The listing builds one solid part. Answer for the finished solid, in the listing's coordinates (mm). Give positions to 0.01 mm unless a question says otherwise; leave off trailing zeros. Write each loop counter-clockwise with the first axis right and the second up, starting at its lowest first coordinate (ties: lowest second). Pieces come first, ordered by that corner, then holes. Notation, with made-up numbers: (-19, -37.75) - (27, -37.75) arc R10 cw to (27, -23.75) - close; hole circle Ø7 at (-1, 52.25). An arc over 180 degrees is marked (long way). Return JSON: item names as keys, results as strings.
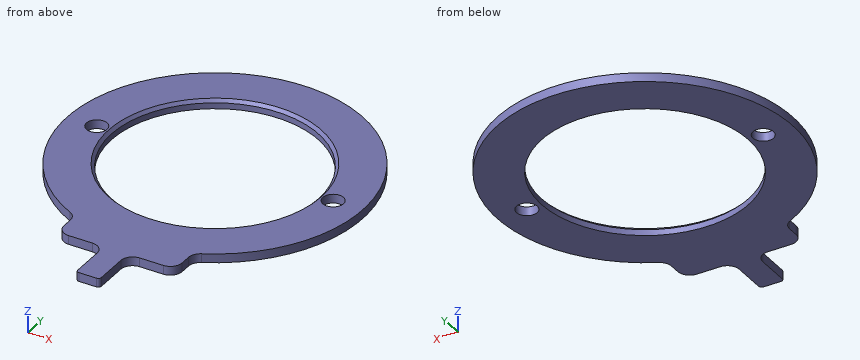
from build123d import *

# Parameters (mm, degrees)
SKETCH_1_R          = 25
SKETCH_1_R_2        = 17.5
EXTRUDE_1_DEPTH     = 1.5
SKETCH_4_W          = 20
SKETCH_4_H          = 15
EXTRUDE_2_DEPTH     = 1.5
SKETCH_5_W          = 8
SKETCH_5_H          = 8
CUT_EXTRUDE_3_DEPTH = 20
FILLET_2_R          = 2
SKETCH_6_R          = 1.75
CUT_EXTRUDE_4_DEPTH = 40
FILLET_3_R          = 0.5
CHAMFER_1_SIZE      = 0.5


with BuildPart() as part:
    # 草图1 → 凸台-拉伸1 (new body)
    with BuildSketch(Plane.XY):
        Circle(SKETCH_1_R)
        Circle(SKETCH_1_R_2, mode=Mode.SUBTRACT)
    extrude(amount=EXTRUDE_1_DEPTH)

    # 草图4 → 凸台-拉伸2 (add)
    with BuildSketch(Plane.XY.offset(1.5)):
        with Locations((0, -28.5)):
            Rectangle(SKETCH_4_W, SKETCH_4_H)
    extrude(amount=-EXTRUDE_2_DEPTH)

    # 草图5 → 切除-拉伸3 (cut)
    with BuildSketch(Plane.XY.offset(1.5)):
        with Locations((-6, -32)):
            Rectangle(SKETCH_5_W, SKETCH_5_H)
        with Locations((6, -32)):
            Rectangle(SKETCH_5_W, SKETCH_5_H)
    extrude(amount=-CUT_EXTRUDE_3_DEPTH, mode=Mode.SUBTRACT)

    # 圆角2
    fillet_2_edges = [part.edges().sort_by_distance(p)[0] for p in [
        (10, -22.912878475, 0.75),
        (-10, -22.912878475, 0.75),
        (-10, -28, 0.75),
        (-2, -28, 0.75),
        (2, -28, 0.75),
        (10, -28, 0.75),
    ]]
    fillet(fillet_2_edges, radius=FILLET_2_R)

    # 草图6 → 切除-拉伸4 (cut)
    with BuildSketch(Plane.XY.offset(1.5)):
        with Locations((-20, 0)):
            Circle(SKETCH_6_R)
        with Locations((20, 0)):
            Circle(SKETCH_6_R)
    extrude(amount=-CUT_EXTRUDE_4_DEPTH, mode=Mode.SUBTRACT)

    # 圆角3
    fillet_3_edges = [part.edges().sort_by_distance(p)[0] for p in [
        (-2, -36, 0.75),
        (2, -36, 0.75),
    ]]
    fillet(fillet_3_edges, radius=FILLET_3_R)

    # 倒角1
    chamfer_1_edges = [part.edges().sort_by_distance(p)[0] for p in [
        (-17.5, 0, 1.5),
    ]]
    chamfer(chamfer_1_edges, length=CHAMFER_1_SIZE)


solid = part.part
Item 1: Consider L1, parallel to X at y = -0.5, z = 0.95 (3 decimals); L2, parallel to X at y = 1.5, z = 1.4; L3, parallel to Y at x = 0, z = 0.8. Determine where each line is inside the solid, lowest interval first.
Answer below:
{"L1": "x = -24.995 to -21.677, -18.323 to -17.493, 17.493 to 18.323, 21.677 to 24.995", "L2": "x = -24.95 to -20.9, -19.1 to -17.84, 17.84 to 19.1, 20.9 to 24.95", "L3": "y = -36 to -17.5, 17.5 to 25"}
Item 2: A cutting plane is placed at D-D on x = -20. Determine the outline of the cut face in (y, z).
Answer below:
{"outline": "(-15, 0) - (-1.75, 0) - (-1.75, 1.5) - (-15, 1.5) - close; (1.75, 0) - (15, 0) - (15, 1.5) - (1.75, 1.5) - close"}
Item 3: A cutting plane is placed at B-B on y = 0. Determine the outline of the cut face in (x, z), then the cut area to 4 significant figures.
Answer below:
{"outline": "(-25, 0) - (-21.75, 0) - (-21.75, 1.5) - (-25, 1.5) - close; (-18.25, 0) - (-17.5, 0) - (-17.5, 1) - (-18, 1.5) - (-18.25, 1.5) - close; (17.5, 0) - (18.25, 0) - (18.25, 1.5) - (18, 1.5) - (17.5, 1) - close; (21.75, 0) - (25, 0) - (25, 1.5) - (21.75, 1.5) - close", "area": "11.75 mm²"}
Item 4: A cutting plane is placed at C-C on z = 0.55. Determine the outline of the cut face in (x, y), then the cut area to 3 significant figures.
Answer below:
{"outline": "(-11.11, -22.4) arc R2 cw to (-10, -24.19) - (-10, -26) arc R2 ccw to (-8, -28) - (-4, -28) arc R2 cw to (-2, -30) - (-2, -35.5) arc R0.5 ccw to (-1.5, -36) - (1.5, -36) arc R0.5 ccw to (2, -35.5) - (2, -30) arc R2 cw to (4, -28) - (8, -28) arc R2 ccw to (10, -26) - (10, -24.19) arc R2 cw to (11.11, -22.4) arc R25 ccw (long way) to start; hole circle Ø3.5 at (-20, 0); hole circle Ø35 at (0, 0); hole circle Ø3.5 at (20, 0)", "area": "1,090 mm²"}
Item 5: A cutting plane is placed at A-A on x = 0. Determine the outline of the cut face in (y, z).
Answer below:
{"outline": "(-36, 0) - (-17.5, 0) - (-17.5, 1) - (-18, 1.5) - (-36, 1.5) - close; (17.5, 0) - (25, 0) - (25, 1.5) - (18, 1.5) - (17.5, 1) - close"}
